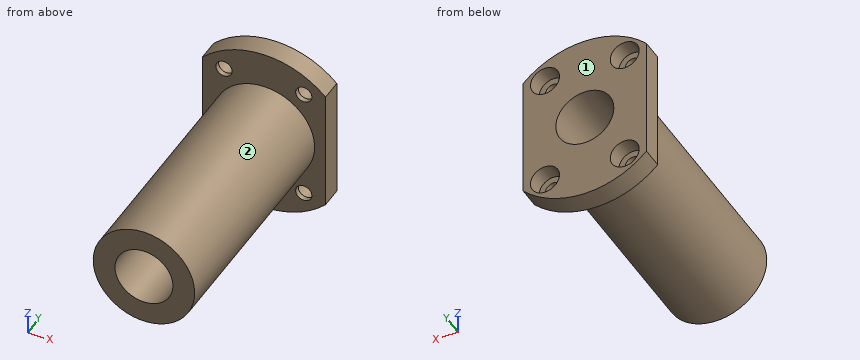
```python
from build123d import *

# Parameters (mm, degrees)
SKETCH1_R                                            = 14
BOSS_EXTRUDE1_DEPTH                                  = 64
SKETCH2_R                                            = 24
BOSS_EXTRUDE2_DEPTH                                  = 6
SKETCH3_OUTSIDE_W                                    = 69.502
SKETCH3_OUTSIDE_H                                    = 69.502
CUT_EXTRUDE2_DEPTH                                   = 6
SKETCH4_R                                            = 8
CUT_EXTRUDE3_DEPTH                                   = 76.927597091
HOLE_SIZE_PER_SOCKET_HEAD_CAP_SCREW_TYPE_D           = 4.5
HOLE_SIZE_PER_SOCKET_HEAD_CAP_SCREW_TYPE_CBORE_D     = 8
HOLE_SIZE_PER_SOCKET_HEAD_CAP_SCREW_TYPE_CBORE_DEPTH = 4.6


with BuildPart() as part:
    # Sketch1 → Boss-Extrude1 (new body)
    with BuildSketch(Plane(origin=(0, 0, 0), x_dir=(1, 0, 0), z_dir=(0, 1, 0))):
        with Locations(Location((0, 0, 0), (0, 0, 270))):
            Circle(SKETCH1_R)
    extrude(amount=BOSS_EXTRUDE1_DEPTH)

    # Sketch2 → Boss-Extrude2 (add)
    with BuildSketch(Plane(origin=(0, 64, 0), x_dir=(1, 0, 0), z_dir=(0, 1, 0))):
        with Locations(Location((0, 0, 0), (0, 0, 270))):
            Circle(SKETCH2_R)
    extrude(amount=BOSS_EXTRUDE2_DEPTH)

    # Sketch3 outside → Cut-Extrude2 (cut)
    with BuildSketch(Plane(origin=(0, 70, 0), x_dir=(1, 0, 0), z_dir=(0, 1, 0))):
        Rectangle(SKETCH3_OUTSIDE_W, SKETCH3_OUTSIDE_H)
        with BuildLine():
            Line((-17, 16.941074346), (-17, -16.941074346))
            ThreePointArc((-17, -16.941074346), (0, -24), (17, -16.941074346))
            Line((17, -16.941074346), (17, 16.941074346))
            ThreePointArc((17, 16.941074346), (0, 24), (-17, 16.941074346))
        make_face(mode=Mode.SUBTRACT)
    extrude(amount=-CUT_EXTRUDE2_DEPTH, mode=Mode.SUBTRACT)

    # Sketch4 → Cut-Extrude3 (cut, through all)
    with BuildSketch(Plane.XZ):
        with Locations(Location((0, 0, 0), (0, 0, 270))):
            Circle(SKETCH4_R)
    extrude(amount=-CUT_EXTRUDE3_DEPTH, mode=Mode.SUBTRACT)

    # Hole size per socket head cap screw type1 (through all)
    with Locations(Plane(origin=(0, 70, 0), x_dir=(-1, 0, 0), z_dir=(0, 1, 0))):
        with Locations((-11, 15.5), (11, 15.5), (11, -15.5), (-11, -15.5)):
            CounterBoreHole(HOLE_SIZE_PER_SOCKET_HEAD_CAP_SCREW_TYPE_D / 2, HOLE_SIZE_PER_SOCKET_HEAD_CAP_SCREW_TYPE_CBORE_D / 2, HOLE_SIZE_PER_SOCKET_HEAD_CAP_SCREW_TYPE_CBORE_DEPTH)


solid = part.part
```
The listing builds one solid part. Answer for the finished solid, in the listing's coordinates (mm). Face numbers are marked on the shaded views. A direction names the side the tool comes from. Coordinates: 2 decimals unless noted, no trailing zeros. Write each loop counter-clockwise with the first axis right and the second up, starting at its lowest first coordinate (ties: lowest second). Pieces come first, ordered by that corner, then holes. Notation, with made-up numbers: M -38,-4.75 L 13,-4.75 A17 cw 13,6.25 Z; hole C 52,17 d6. An arc over 180 degrees is marked long. Use a Markdown table: item, result. Add a question column.
1. Which of the six approach directions +Z, -Z, +X, -X, +Y, -Y give full straight-line access (tool end or side, diameter ignored) to the marked faces 1 and 2?
2. Section B-B (x = 0) is taken. Give the vertices of the cut face in (y, z).
3. Section A-A (z = 15.5) is taken. Give the vertices of the cut face in (x, y), plus the area to 3 significant figures.
4. Section C-C (y = 20.5) is taken. Give the vertices of the cut face in (x, z), plus the area to 3 significant figures.
5. Section D-D (x = 11) is taken. Give the vertices of the cut face in (y, z).
6. Straight lines are drawn through the part: line 1 along X through (y, z) = (26.5, 0); line 2 along X through (y, z) = (66, -15); line 3 along Z through (x, y) = (-11, 64.75). For each, find the intervals that lie inside material, in ascending order. Write a range as [from, to].
7. Given P1, Ø9, axis at x = 10, z = 16.5, coming from the +Y side; P2, Ø6.5, axis at x = 11, z = 15.5, coming from the +Y side; P3, Ø4, axis at x = -7.5, y = 38, coming from the +Z side; P4, Ø7, axis at x = 11, z = -15.5, coming from the -Y side, each flat-ended and moving along its own axis, determine where each tip first touches the part or whether it passes through.
Data:
| question | item | result |
|---|---|---|
| 1 | face 1 | +Z, -Z, +X, -X, +Y |
| 1 | face 2 | -Y |
| 2 | outline | M 0,-14 L 64,-14 L 64,-24 L 70,-24 L 70,-8 L 0,-8 Z; M 0,8 L 70,8 L 70,24 L 64,24 L 64,14 L 0,14 Z |
| 3 | outline | M -17,64 L -13.25,64 L -13.25,65.4 L -15,65.4 L -15,70 L -17,70 Z; M -8.75,64 L 8.75,64 L 8.75,65.4 L 7,65.4 L 7,70 L -7,70 L -7,65.4 L -8.75,65.4 Z; M 13.25,64 L 17,64 L 17,70 L 15,70 L 15,65.4 L 13.25,65.4 Z |
| 3 | area | 118 mm2 |
| 4 | outline | C 0,0 d28; hole C 0,0 d16 |
| 4 | area | 415 mm2 |
| 5 | outline | M 0,-8.66 L 64,-8.66 L 64,-13.25 L 65.4,-13.25 L 65.4,-11.5 L 70,-11.5 L 70,11.5 L 65.4,11.5 L 65.4,13.25 L 64,13.25 L 64,8.66 L 0,8.66 Z; M 64,-21.33 L 70,-21.33 L 70,-19.5 L 65.4,-19.5 L 65.4,-17.75 L 64,-17.75 Z; M 64,17.75 L 65.4,17.75 L 65.4,19.5 L 70,19.5 L 70,21.33 L 64,21.33 Z |
| 6 | line 1 | x = [-14, -8], [8, 14] |
| 6 | line 2 | x = [-17, -14.97], [-7.03, 7.03], [14.97, 17] |
| 6 | line 3 | z = [-21.33, -17.75], [-13.25, 13.25], [17.75, 21.33] |
| 7 | P1 | stops at y = 70 |
| 7 | P2 | stops at y = 65.4 |
| 7 | P3 | stops at z = 12.87 |
| 7 | P4 | stops at y = 64 |
